Answer from the drawing. Dimensions are ordinates in mm from the lowest x, y and z of the part. Coordinates: 2 decimals unless noted, no trailing zeros. Write each loop counter-clockwise with the first axis right and the second up, starting at its lowest first coordinate (ties: lowest second). Pieces come first, ordered by that corner, then holes.
1) The part is cut by section B-B (y = 13.25). Determine the outline of the cut face in (x, z), then the cut area to 3 significant figures.
2) The part is cut by section A-A (x = 12). Determine the outline of the cut face in (y, z) (1 decimal).
3) Find the intervals of material crossed by line 1 (Z direction, x = 4, y = 6.75); line 2 (Y direction, x = 12.25, z = 53); line 3 (X direction, y = 11, z = 46), in increasing order.
4) Each of these flat-tipped pins is pushed along its axis until it touches: pin 1 Ø10 at (y, z) = (17, 28) entering from +X; pin 2 Ø10 at (x, z) = (12, 80) entering from +Y; pin 3 Ø12 at (y, z) = (6.5, 178.5) entering from -X. Where does it stop, or does it pass through?
5) The part is cut by section C-C (z = 57). Determine the outline of the cut face in (x, y).
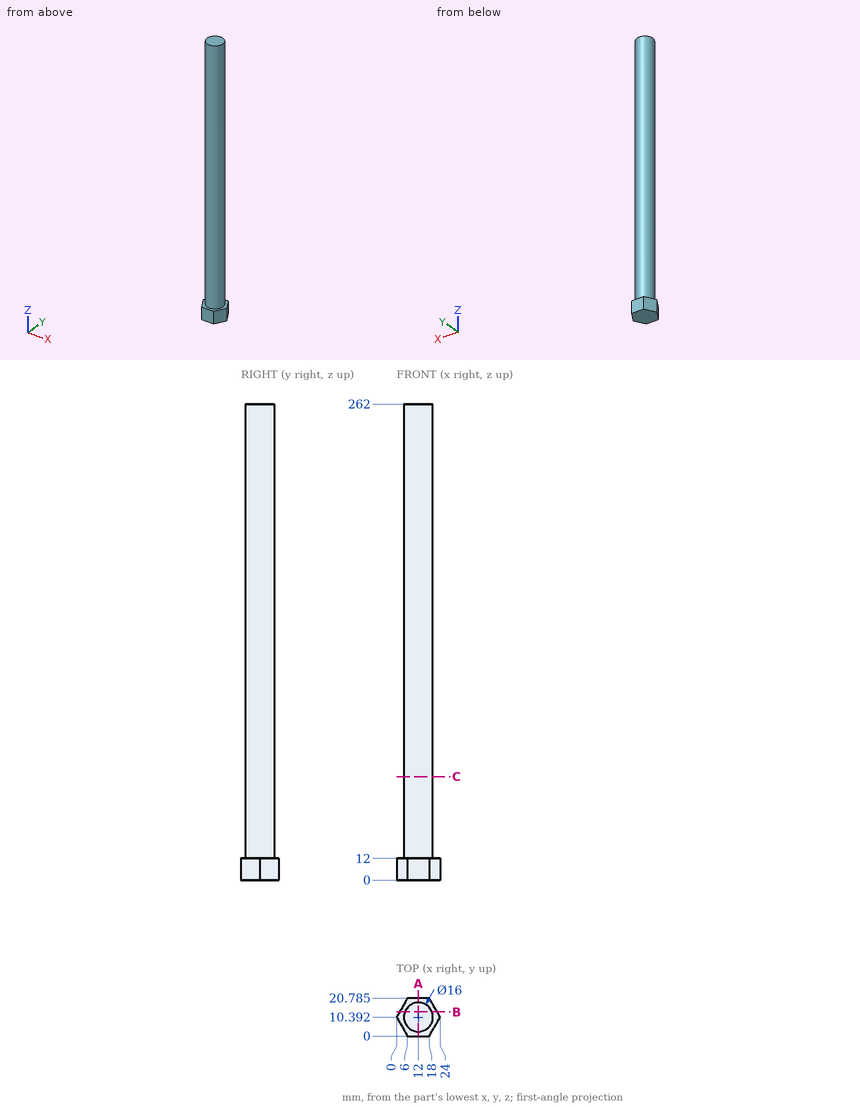
Reported:
1. outline: (1.65, 0) - (22.35, 0) - (22.35, 12) - (19.47, 12) - (19.47, 262) - (4.53, 262) - (4.53, 12) - (1.65, 12) - close
1. area: 3,980 mm2
2. outline: (0, 0) - (20.8, 0) - (20.8, 12) - (18.4, 12) - (18.4, 262) - (2.4, 262) - (2.4, 12) - (0, 12) - close
3. line 1: z = 0 to 12
3. line 2: y = 2.4 to 18.39
3. line 3: x = 4.02 to 19.98
4. pin 1: stops at x = 19.84
4. pin 2: stops at y = 18.39
4. pin 3: stops at x = 4
5. outline: circle Ø16 at (12, 10.39)
